The drawing under review shows one solid part. Ordinate dimensions are in mm from its lowest x, y, z. A direction names the side the tool comes from. Round coordinates to 2 decimals unless told otherwise and drop trailing zeros. Write each loop counter-clockwise with the first axis right and the second up, starting at its lowest first coordinate (ties: lowest second). Pieces come first, ordered by that corner, then holes. Notation, with made-up numbers: (70, 80) -> (76, 80) arc R28 cw to (76, 118) -> close; hole circle Ø10 at (48.25, 44). An arc over 180 degrees is marked (long way). Answer in a Markdown table with one row per item. Add a question column.
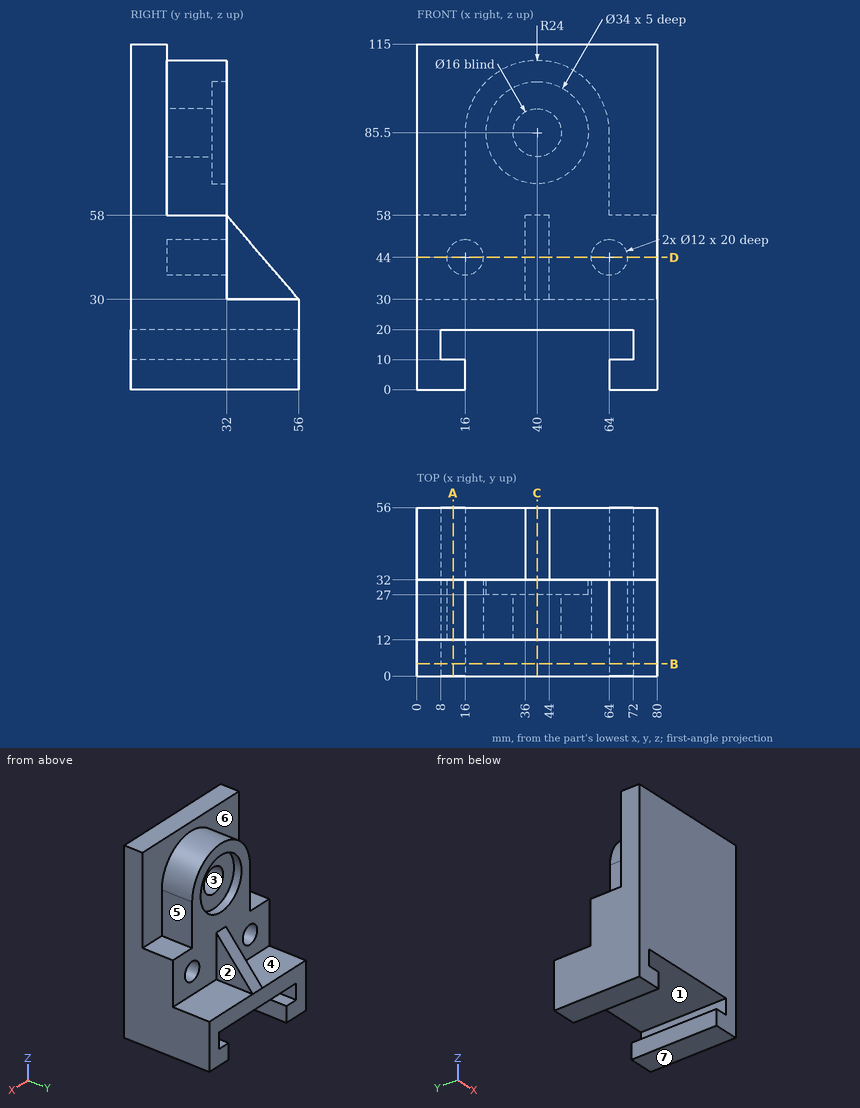
1. For L1, parallel to X at y = 21, z = 44; L2, parallel to Z at x = 11, y = 24; L3, parallel to X at y = 34, z = 54, list the stretches that pass through material, from the lowest coordinate up.
2. Add section C-C on x = 40. Write out the cut boundary in (y, z), plus the area to 3 significant figures.
3. Insertion check: pin 1 Ø10 at (y, z) = (27, 67.5) entering from -X; pin 2 Ø19 at (x, y) = (69, 48.5) entering from +Z; pin 3 Ø3.5 at (x, z) = (62, 42) entering from +Y. Each pin has a flat end and moves straight along its axis. Give the tip position at first contact, or say it passes through.
4. Add section D-D on z = 44. Write out the cut boundary in (x, y).
5. Tool access review of the marked faces 5, 6 and 7: name each direction out of +Z, -Z, +X, -X, +Y, -Y from which nothing blocks a thin tool from reaching the whole face with its end or side.
6. Add section B-B on y = 4. Write out the cut boundary in (x, z), plus the area to 3 significant figures.
7. Mouldability with a two-part tool opening along X and no side actions: class the marked faces 1, 2, 3 and 4 as pulls with the +X half, pulls with the -X half, needs draft (parallel to the pull), parting line crosses it, or undercut.
8. Add section A-A on x = 12. Write out the cut boundary in (y, z).
Filled in:
| question | item | result |
|---|---|---|
| 1 | L1 | 0 to 10, 22 to 58, 70 to 80 |
| 1 | L2 | 0 to 10, 20 to 40.68, 47.32 to 58 |
| 1 | L3 | 36 to 44 |
| 2 | outline | (0, 20) -> (56, 20) -> (56, 30) -> (32, 58) -> (32, 68.5) -> (27, 68.5) -> (27, 77.5) -> (12, 77.5) -> (12, 93.5) -> (27, 93.5) -> (27, 102.5) -> (32, 102.5) -> (32, 109.5) -> (12, 109.5) -> (12, 115) -> (0, 115) -> close |
| 2 | area | 3,100 mm² |
| 3 | pin 1 | x = 16 |
| 3 | pin 2 | z = 30 |
| 3 | pin 3 | y = 12 |
| 4 | outline | (0, 0) -> (80, 0) -> (80, 32) -> (70, 32) -> (70, 12) -> (58, 12) -> (58, 32) -> (44, 32) -> (44, 44) -> (36, 44) -> (36, 32) -> (22, 32) -> (22, 12) -> (10, 12) -> (10, 32) -> (0, 32) -> close |
| 5 | face 5 | +Z, +X, +Y |
| 5 | face 6 | +Z, +Y |
| 5 | face 7 | -Z, +X, -X, +Y, -Y |
| 6 | outline | (0, 0) -> (16, 0) -> (16, 10) -> (8, 10) -> (8, 20) -> (72, 20) -> (72, 10) -> (64, 10) -> (64, 0) -> (80, 0) -> (80, 115) -> (0, 115) -> close |
| 6 | area | 8,080 mm² |
| 7 | face 1 | undercut |
| 7 | face 2 | pulls with the +X half |
| 7 | face 3 | undercut |
| 7 | face 4 | needs draft |
| 8 | outline | (0, 0) -> (56, 0) -> (56, 10) -> (0, 10) -> close; (0, 20) -> (56, 20) -> (56, 30) -> (32, 30) -> (32, 39.53) -> (12, 39.53) -> (12, 48.47) -> (32, 48.47) -> (32, 58) -> (12, 58) -> (12, 115) -> (0, 115) -> close |
